Verification items for the finished model (mm, model axes). Round coordinates to 2 decimals unless told otherwise and drop trailing zeros. Write each loop counter-clockwise with the first axis right and the second up, starting at its lowest first coordinate (ties: lowest second). Pieces come first, ordered by that corner, then holes.
from build123d import *

# Parameters (mm, degrees)
SKETCH_1_W             = 10
SKETCH_1_H             = 240
EXTRUDE_1_DEPTH        = 50
HOLE_WIZARD_M4_2_D     = 3.3
HOLE_WIZARD_M4_2_DEPTH = 15
HOLE_WIZARD_M4_2_TIP   = 0.991420021
HOLE_WIZARD_M4_3_D     = 3.3
HOLE_WIZARD_M4_3_DEPTH = 15
HOLE_WIZARD_M4_3_TIP   = 0.991420021
CHAMFER_1_SIZE         = 30
CHAMFER_1_SIZE2        = 60


with BuildPart() as part:
    # 草图1 → 凸台-拉伸1 (new body)
    with BuildSketch(Plane.XY):
        Rectangle(SKETCH_1_W, SKETCH_1_H)
    extrude(amount=EXTRUDE_1_DEPTH)

    # M4 螺纹孔2
    with Locations(Plane(origin=(0, 0, 0), x_dir=(-1, 0, 0), z_dir=(0, 0, -1))):
        with Locations((0, 97.5), (0, 32.5), (0, -32.5), (0, -97.5)):
            Hole(HOLE_WIZARD_M4_2_D / 2, depth=HOLE_WIZARD_M4_2_DEPTH)
            with Locations((0, 0, -(HOLE_WIZARD_M4_2_DEPTH + HOLE_WIZARD_M4_2_TIP / 2))):  # 118° drill point
                Cone(0, HOLE_WIZARD_M4_2_D / 2, HOLE_WIZARD_M4_2_TIP, mode=Mode.SUBTRACT)

    # M4 螺纹孔3
    with Locations(Plane(origin=(0, -120, 0), x_dir=(-1, 0, 0), z_dir=(0, -1, 0))):
        with Locations((0, -10), (0, -40)):
            Hole(HOLE_WIZARD_M4_3_D / 2, depth=HOLE_WIZARD_M4_3_DEPTH)
            with Locations((0, 0, -(HOLE_WIZARD_M4_3_DEPTH + HOLE_WIZARD_M4_3_TIP / 2))):  # 118° drill point
                Cone(0, HOLE_WIZARD_M4_3_D / 2, HOLE_WIZARD_M4_3_TIP, mode=Mode.SUBTRACT)

    # 倒角1
    chamfer_1_edges = [part.edges().sort_by_distance(p)[0] for p in [
        (0, 120, 50),
    ]]
    chamfer_1_side = [part.faces().sort_by_distance(p)[0] for p in [
        (0, 120, 25),
    ]]
    chamfer(chamfer_1_edges, length=CHAMFER_1_SIZE, length2=CHAMFER_1_SIZE2, reference=chamfer_1_side[0])


solid = part.part
Q1. Material ranges on line 1 along Z through (x, y) = (0, -115.5); line 2 along Y through (x, z) = (0, 3); line 3 along X through (y, z) = (-97.5, 11.5), recorded low to high.
Recorded:
line 1: z = 0 to 8.35, 11.65 to 38.35, 41.65 to 50
line 2: y = -120 to -99.15, -95.85 to -34.15, -30.85 to 30.85, 34.15 to 95.85, 99.15 to 120
line 3: x = -5 to -1.65, 1.65 to 5
Q2. Depth check by flat-ended pin: P1, Ø3, axis at x = 0, z = 40, coming from the -Y side; P2, Ø5.5, axis at x = 0, y = 97.5, coming from the +Z side (3 decimals); P3, Ø5, axis at x = -3, z = 23.5, coming from the +Y side. Enter the tip coordinate at first touch or a pass-through.
Recorded:
P1: stops at y = -104.91
P2: stops at z = 32.625
P3: stops at y = 118
Q3. Sectioned sample at A-A (z = 30). Enter the section's corners in (x, y), plus the area to 3 significant figures.
Recorded:
outline: (-5, -120) - (5, -120) - (5, 100) - (-5, 100) - close
area: 2,200 mm2
Q4. Release check for a two-part mould opening along Z. For faces 1 (the flat face through (0, 2, 0)), 2 (the flat face through (5, -2, 25)), 3 (the flat face through (0, -29, 50)) record: released by +Z, released by -Z, zero draft, split by the parting line, or undercut.
Recorded:
face 1: released by -Z
face 2: zero draft
face 3: released by +Z
